from build123d import *

# Parameters (mm, degrees)
SKETCH2_R          = 9.5
CUT_EXTRUDE1_DEPTH = 70
CHAMFER1_SIZE      = 1
SKETCH7_W          = 6
SKETCH7_H          = 6
CUT_EXTRUDE2_DEPTH = 70


with BuildPart() as part:
    # Sketch1 → Revolve1 (revolve)
    with BuildSketch(Plane.XY):
        Polygon((0, 0), (0, 50), (3, 50), (7.003672577, 39), (15.996327423, 39), (20, 50), (22, 50), (26.003672577, 39), (34.996327423, 39), (39, 50), (42, 50), (42, 30), (54, 30), (54, 0), align=None)
    revolve(axis=Axis((54, 0, 0), (-1, 0, 0)))

    # Sketch2 → Cut-Extrude1 (cut)
    with BuildSketch(Plane(origin=(54, 0, 0), x_dir=(0, 0, -1), z_dir=(1, 0, 0))):
        with Locations(Location((0, 0, 0), (0, 0, 90))):
            Circle(SKETCH2_R)
    extrude(amount=-CUT_EXTRUDE1_DEPTH, mode=Mode.SUBTRACT)

    # Sketch5 → M6 Tapped Hole1 (revolve, cut)
    with BuildSketch(Plane.YZ.offset(46.5)):
        Polygon((0, 0), (0, 51.502151548), (2.5, 50), (2.5, 0), align=None)
    revolve(axis=Axis((46.5, 0, -6.35), (0, 0, 1)), mode=Mode.SUBTRACT)

    # Chamfer1
    chamfer1_edges = [part.edges().sort_by_distance(p)[0] for p in [
        (54, -30, 0),
    ]]
    chamfer(chamfer1_edges, length=CHAMFER1_SIZE)

    # Sketch7 → Cut-Extrude2 (cut)
    with BuildSketch(Plane(origin=(54, 0, 0), x_dir=(0, 0, -1), z_dir=(1, 0, 0))):
        with Locations((-9.5, 0)):
            Rectangle(SKETCH7_W, SKETCH7_H)
    extrude(amount=-CUT_EXTRUDE2_DEPTH, mode=Mode.SUBTRACT)


solid = part.part
The listing builds one solid part. Answer for the finished solid, in the listing's coordinates (mm). A direction names the side the tool comes from. Give positions to 0.01 mm unless a question says otherwise; leave off trailing zeros. Write each loop counter-clockwise with the first axis right and the second up, starting at its lowest first coordinate (ties: lowest second). Pieces come first, ordered by that corner, then holes.
1) Given P1, Ø1, axis at y = -32.5, z = 23.5, coming from the +X side; P2, Ø1.8, axis at x = 14, y = 0, coming from the -Z side; P3, Ø1, axis at x = 41, z = -19, coming from the +Y side; P4, Ø24.5, axis at y = 0, z = 0, coming from the +X side, each flat-ended and moving along its own axis, determine where each tip first touches the part or whether it passes through.
2) Find the intervals of material crossed by L1, parallel to X at y = 0, z = 44; L2, parallel to Y at x = 31, z = 0; L3, parallel to X at y = 0, z = 20, in increasing order.
3) For a pull along X with two mould halves and no side action, classify faces 6 (the face through (6.81, 18.24, 35.07)), 7 (the face through (54, -7, -7)), 8 (the face through (21.01, 47.69, -15.02)) as pulls with the +X half, pulls with the -X half, needs draft (parallel to the pull), parting line crosses it, or undercut.
4) Section A-A (y = 0) is taken. Count the separate pieces of the cut face and the enclosed holes in it, and give its area (3 significant figures).
5) Section C-C (x = 46.5) is taken. Write down the section's boundary in (y, z), and give its area (3 significant figures).
6) A tool of negligible diameter and unlimited length cuts with its end or side. For faces 1 (the face through (0, -10, -1)), 2 (the face through (16.247, 18.314, 35.21)), 3 (the face through (42, 22, 22)), 4 (the face through (27, -3, 11)), 5 (the face through (48.94, -0.54, 21.13)), from which of +Z, -Z, +X, -X, +Y, -Y can it reach the whole face along a straight path? Write none if from no direction.
Response:
1. P1: stops at x = 42
1. P2: stops at z = -39
1. P3: stops at y = 46.45
1. P4: stops at x = 54
2. L1: x = 0 to 5.18, 17.82 to 24.18, 36.82 to 42
2. L2: y = -39 to -9.5, 9.5 to 39
2. L3: x = 0 to 44, 49 to 54
3. face 6: undercut
3. face 7: pulls with the +X half
3. face 8: needs draft
4. separate pieces: 3
4. enclosed holes: 0
4. area: 3,070 mm2
5. outline: (-3, 9.01) - (-3, 12.5) - (-2.5, 12.5) - (-2.5, 29.9) arc R30 ccw (long way) to (2.5, 29.9) - (2.5, 12.5) - (3, 12.5) - (3, 9.01) arc R9.5 cw (long way) to start
5. area: 2,440 mm2
6. face 1: +Z, -Z, -X, +Y, -Y
6. face 2: none
6. face 3: +X
6. face 4: +X, -X
6. face 5: +Z
